Could you check a few things on this drawing? It's one solid part, dimensions in mm from its lowest x, y, z. Round coordinates to 2 decimals unless told otherwise and drop trailing zeros. Loops run counter-clockwise (first coordinate to the right, second up) from the corner with the lowest first, then second, coordinate; pieces in that order, holes last.
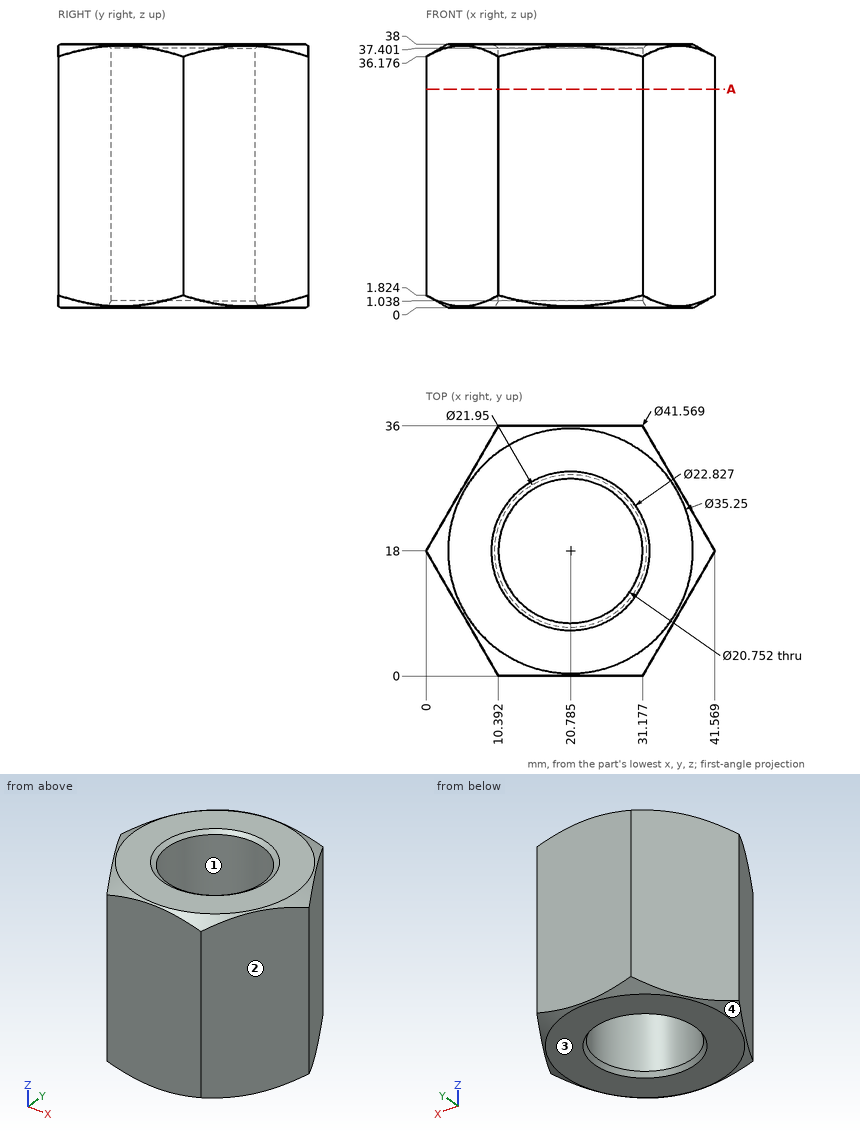
(1) We'd pull the mould along Y, two halves only. Please class the marked faces 1, 2, 3 and 4: released by +Y, released by -Y, zero draft, split by the parting line, or undercut.
(2) Suppose I cut it at A-A (z = 31.5). Write out the boundary of the cut face in (x, y) (1 decimal).
(3) For pin 1 (1.5 mm diameter, centred on y = 3.5, z = 13, fed in from +X); pin 2 (12.5 mm diameter, centred on x = 20.78, y = 18, fed in from +Z); pin 3 (1 mm diameter, centred on y = 6, z = 11, fed in from +X); pin 4 (6 mm diameter, centred on y = 22.5, z = 30, fed in from -X) (1 decimal), each with a flat end and sliding along its axis, tell me the tip position at first contact or that it passes through.
(4) If I drill on line 1 (Y direction, x = 19.5, z = 31); line 2 (X direction, y = 14.5, z = 18); line 3 (Y direction, x = 28, z = 23) (1 decimal), over which ranges is the centre line in solid material (lowest first)?
Check result:
1. face 1: undercut
1. face 2: released by -Y
1. face 3: zero draft
1. face 4: split by the parting line
2. outline: (0, 18) - (10.4, 0) - (31.2, 0) - (41.6, 18) - (31.2, 36) - (10.4, 36) - close; hole circle Ø20.8 at (20.8, 18)
3. pin 1: stops at x = 33.63
3. pin 2: passes through
3. pin 3: stops at x = 34.93
3. pin 4: stops at x = 0.9
4. line 1: y = 0 to 7.7, 28.3 to 36
4. line 2: x = 2.02 to 11.02, 30.55 to 39.55
4. line 3: y = 0 to 10.5, 25.5 to 36
